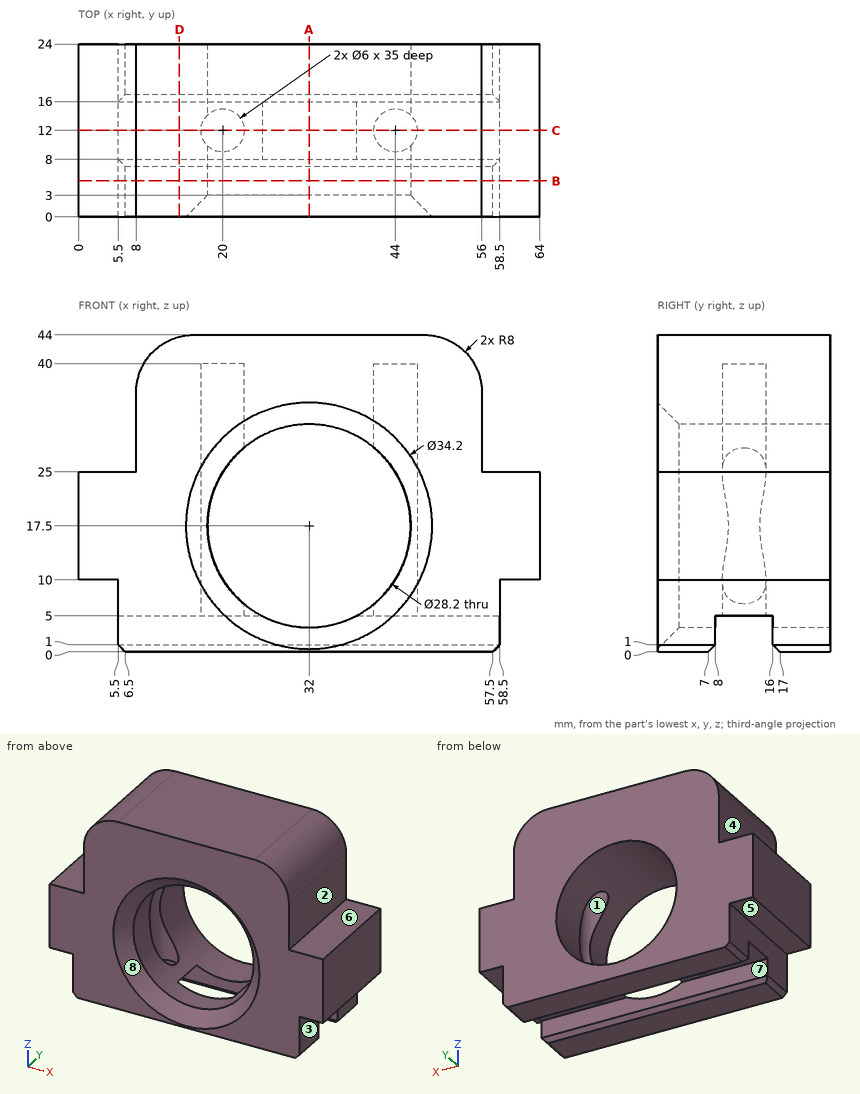
Source: three-view drawing plus pictorial views. Frame: mm from the lowest corner of the part. A direction names the side the tool comes from. Round coordinates to 2 decimals unless told otherwise and drop trailing zeros. Order: outer loops, then holes, each group sorted by start corner. A loop starts at its lowest first (then second) coordinate and runs counter-clockwise, first axis right, second up. Notation, with made-up numbers: (33.25, -7.5) - (74.25, -7.5) arc R16 cw to (74.25, 11.5) - close; hole circle Ø10 at (49.5, 31.5). An arc over 180 degrees is marked (long way). Answer in a Markdown table with one row per item.
Item 1: Reachability of the marked faces 1, 2, 3, 4 and 5 from +Z, -Z, +X, -X, +Y, -Y: full face, straight path, thin tool, end or side. Return the list, or none.
Model answer:
| item | result |
|---|---|
| face 1 | -Z |
| face 2 | +Z, +X, +Y, -Y |
| face 3 | -Z, +X, +Y, -Y |
| face 4 | +Z, -X, +Y, -Y |
| face 5 | -Z, -X, +Y, -Y |
Item 2: Section query B-B (y = 5). Return the cut outline in (x, z), then the cut area to 3 significant figures.
Model answer:
| item | result |
|---|---|
| outline | (0, 10) - (5.5, 10) - (5.5, 1) - (6.5, 0) - (57.5, 0) - (58.5, 1) - (58.5, 10) - (64, 10) - (64, 25) - (56, 25) - (56, 36) arc R8 ccw to (48, 44) - (16, 44) arc R8 ccw to (8, 36) - (8, 25) - (0, 25) - close; hole circle Ø28.2 at (32, 17.5) |
| area | 1,750 mm² |
Item 3: Pin query (flat end, axial travel): pin 1 (12 mm diameter, centred on y = 7.5, z = 32.5, fed in from +X); pin 2 (4 mm diameter, centred on x = 60.5, y = 8.5, fed in from +Z); pin 3 (2 mm diameter, centred on x = 25.5, z = 4, fed in from -Y). Return the tip coordinate at first contact, or that it passes through.
Model answer:
| item | result |
|---|---|
| pin 1 | stops at x = 56 |
| pin 2 | stops at z = 25 |
| pin 3 | stops at y = 1.12 |
Item 4: Section query A-A (x = 32). Return the cut outline in (y, z), then the cut area to 3 significant figures.
Model answer:
| item | result |
|---|---|
| outline | (0, 0) - (7, 0) - (8, 1) - (8, 3.4) - (3, 3.4) - (0, 0.4) - close; (0, 34.6) - (3, 31.6) - (24, 31.6) - (24, 44) - (0, 44) - close; (16, 1) - (17, 0) - (24, 0) - (24, 3.4) - (16, 3.4) - close |
| area | 342 mm² |
Item 5: Line query: line 1 (X direction, y = 15.75, z = 17.5); line 2 (Z direction, x = 23, y = 18.25); line 3 (X direction, y = 22.5, z = 32.5). Output: solid intervals per line, ascending.
Model answer:
| item | result |
|---|---|
| line 1 | x = 0 to 17.9, 46.1 to 64 |
| line 2 | z = 0 to 6.65, 28.35 to 44 |
| line 3 | x = 8 to 56 |
Item 6: Section query D-D (x = 14). Return the cut outline in (y, z).
Model answer:
| item | result |
|---|---|
| outline | (0, 0) - (7, 0) - (8, 1) - (8, 5) - (16, 5) - (16, 1) - (17, 0) - (24, 0) - (24, 43.75) - (0, 43.75) - close |
Item 7: Mould query, pull axis Z, two halves, no side actions, for the marked faces 6, 7 and 8. Classes: released by +Z, released by -Z, zero draft, split by the parting line, or undercut.
Model answer:
| item | result |
|---|---|
| face 6 | released by +Z |
| face 7 | zero draft |
| face 8 | undercut |
Item 8: Section query C-C (y = 12). Return the cut outline in (x, z), then the cut area to 3 significant figures.
Model answer:
| item | result |
|---|---|
| outline | (0, 10) - (5.5, 10) - (5.5, 5) - (17, 5) - (17, 40) - (23, 40) - (23, 28.35) arc R14.1 cw to (41, 28.35) - (41, 40) - (47, 40) - (47, 5) - (58.5, 5) - (58.5, 10) - (64, 10) - (64, 25) - (56, 25) - (56, 36) arc R8 ccw to (48, 44) - (16, 44) arc R8 ccw to (8, 36) - (8, 25) - (0, 25) - close; (23, 5) - (25.48, 5) arc R14.1 cw to (23, 6.65) - close; (38.52, 5) - (41, 5) - (41, 6.65) arc R14.1 cw to start |
| area | 1,230 mm² |
